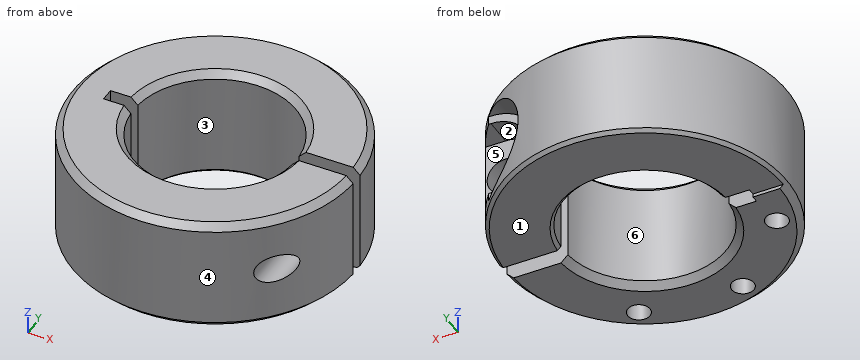
```python
from build123d import *

# Parameters (mm, degrees)
SKETCH2_R             = 21
SKETCH2_R_2           = 12
BOSS_EXTRUDE2_DEPTH   = 17
CHAMFER1_SIZE         = 1
SKETCH3_W             = 46.185652856
SKETCH3_H             = 2
CUT_EXTRUDE1_DEPTH    = 35.219877265
SKETCH5_R             = 2.75
CUT_EXTRUDE3_DEPTH    = 30
CUT_EXTRUDE4_START    = -8
CUT_EXTRUDE4_DEPTH    = 30
M5_TAPPED_HOLE1_D     = 4.2
SKETCH9_W             = 59.171214414
SKETCH9_H             = 29.501144874
CUT_EXTRUDE5_DEPTH    = 0.5
M4_TAPPED_HOLE1_D     = 3.3
M4_TAPPED_HOLE1_DEPTH = 10.1
M4_TAPPED_HOLE1_TIP   = 0.991420021
SKETCH13_R            = 7
CUT_EXTRUDE7_DEPTH    = 17


with BuildPart() as part:
    # Sketch2 → Boss-Extrude2 (new body)
    with BuildSketch(Plane.XY):
        Circle(SKETCH2_R)
        Circle(SKETCH2_R_2, mode=Mode.SUBTRACT)
    extrude(amount=BOSS_EXTRUDE2_DEPTH)

    # Chamfer1
    chamfer1_edges = [part.edges().sort_by_distance(p)[0] for p in [
        (-21, 0, 0),
        (-21, 0, 17),
        (-12, 0, 0),
        (-12, 0, 17),
    ]]
    chamfer(chamfer1_edges, length=CHAMFER1_SIZE)

    # Sketch3 → Cut-Extrude1 (cut, through all)
    with BuildSketch(Plane.XY.offset(17)):
        with Locations((7.092826428, 0)):
            Rectangle(SKETCH3_W, SKETCH3_H)
    extrude(amount=-CUT_EXTRUDE1_DEPTH, mode=Mode.SUBTRACT)

    # Sketch5 → Cut-Extrude3 (cut)
    with BuildSketch(Plane.XZ.offset(-1)):
        with Locations(Location((15.988088482, 8.75, 0), (0, 0, 270))):
            Circle(SKETCH5_R)
    extrude(amount=-CUT_EXTRUDE3_DEPTH, mode=Mode.SUBTRACT)

    # Sketch6 → Cut-Extrude4 (cut)
    with BuildSketch(Plane.XZ.offset(-1).offset(CUT_EXTRUDE4_START)):
        with BuildLine():
            Line((15.988088482, 14.5), (20.976176963, 14.5))
            Line((20.976176963, 14.5), (20.976176963, 3))
            Line((20.976176963, 3), (15.988088482, 3))
            ThreePointArc((15.988088482, 3), (10.238088482, 8.75), (15.988088482, 14.5))
        make_face()
    extrude(amount=-CUT_EXTRUDE4_DEPTH, mode=Mode.SUBTRACT)

    # M5 Tapped Hole1 (through all)
    with Locations(Plane(origin=(0, -1, 0), x_dir=(1, 0, 0), z_dir=(0, 1, 0))):
        with Locations((15.988088482, -8.75)):
            Hole(M5_TAPPED_HOLE1_D / 2)

    # Sketch9 → Cut-Extrude5 (cut)
    with BuildSketch(Plane(origin=(0, 0, 0), x_dir=(-1, 0, 0), z_dir=(0, 0, -1))):
        with Locations((-1.080150951, 14.750572437)):
            Rectangle(SKETCH9_W, SKETCH9_H)
    extrude(amount=-CUT_EXTRUDE5_DEPTH, mode=Mode.SUBTRACT)

    # M4 Tapped Hole1
    with Locations(Plane(origin=(0, 0, 0), x_dir=(-1, 0, 0), z_dir=(0, 0, -1))):
        with Locations((16.444620864, -5.985352508), (-8.75, -15.155444566), (5.985352508, -16.444620864)):
            Hole(M4_TAPPED_HOLE1_D / 2, depth=M4_TAPPED_HOLE1_DEPTH)
            with Locations((0, 0, -(M4_TAPPED_HOLE1_DEPTH + M4_TAPPED_HOLE1_TIP / 2))):  # 118° drill point
                Cone(0, M4_TAPPED_HOLE1_D / 2, M4_TAPPED_HOLE1_TIP, mode=Mode.SUBTRACT)

    # Sketch13 → Cut-Extrude7 (cut)
    with BuildSketch(Plane(origin=(0, 13.2, 0), x_dir=(1, 0, 0), z_dir=(0, 1, 0))):
        with Locations((15.988088482, -8.75)):
            Circle(SKETCH13_R)
    extrude(amount=CUT_EXTRUDE7_DEPTH, mode=Mode.SUBTRACT)


solid = part.part
```
Can you work these out from the model? Positions are in its coordinate system, mm. Face numbers are marked on the shaded views. A direction names the side the tool comes from. Round coordinates to 2 decimals unless told otherwise and drop trailing zeros. Loops run counter-clockwise (first coordinate to the right, second up) from the corner with the lowest first, then second, coordinate; pieces in that order, holes last. Notation, with made-up numbers: (-13.5, 40) -> (43.5, 40) arc R24 ccw to (43.5, 77) -> close; hole circle Ø1 at (11.25, 68). An arc over 180 degrees is marked (long way). Answer in a Markdown table with one row per item.
Item 1: Suppose I cut it at B-B, the plane z = 8.75. List the corners of the cut face in (x, y) for me, plus the area to 3 significant figures.
Answer block:
| item | result |
|---|---|
| outline | (-16, -1) -> (-16, 1) -> (-11.96, 1) arc R12 cw to (11.96, 1) -> (13.24, 1) -> (13.24, 9) -> (10.24, 9) -> (10.24, 13.2) -> (8.99, 13.2) -> (8.99, 18.98) arc R21 ccw (long way) to (13.89, -15.75) -> (13.89, -1) -> (11.96, -1) arc R12 cw to (-11.96, -1) -> close; (18.09, -10.67) arc R21 ccw to (20.98, -1) -> (18.09, -1) -> close; (18.74, 1) -> (20.98, 1) arc R21 ccw to (18.97, 9) -> (18.74, 9) -> close; hole circle Ø3.3 at (-16.44, -5.99); hole circle Ø3.3 at (-5.99, -16.44); hole circle Ø3.3 at (8.75, -15.16) |
| area | 729 mm² |
Item 2: We'd pull the mould along X, two halves only. Please class the marked faces 4, 5 and 6: released by +X, released by -X, zero draft, split by the parting line, or undercut.
Answer block:
| item | result |
|---|---|
| face 4 | split by the parting line |
| face 5 | zero draft |
| face 6 | undercut |
Item 3: If I drill on probe 1 along Y at (x, z) = (-5.5, 4.5); probe 2 along Y at (x, z) = (-15.5, 8.5); probe 3 along X at (y, z) = (3.5, 10.75), over which ranges is the centre line in solid material (lowest first)?
Answer block:
| item | result |
|---|---|
| probe 1 | -20.27 to -18.02, -14.87 to -10.67, 10.67 to 20.27 |
| probe 2 | -14.17 to -7.34, -4.63 to -1, 1 to 14.17 |
| probe 3 | -20.71 to -11.48, 11.48 to 14.1, 17.88 to 20.71 |
Item 4: Suppose I cut it at A-A, the plane x = 0. List the corners of the cut face in (y, z) for me.
Answer block:
| item | result |
|---|---|
| outline | (-21, 1) -> (-20, 0) -> (-13, 0) -> (-12, 1) -> (-12, 16) -> (-13, 17) -> (-20, 17) -> (-21, 16) -> close; (12, 1) -> (12.5, 0.5) -> (20.5, 0.5) -> (21, 1) -> (21, 16) -> (20, 17) -> (13, 17) -> (12, 16) -> close |
Item 5: Suppose I cut it at C-C, the plane z = 12.25. List the corners of the cut face in (x, y) for me, plus the area to 3 significant figures.
Answer block:
| item | result |
|---|---|
| outline | (-16, -1) -> (-16, 1) -> (-11.96, 1) arc R12 cw to (11.96, 1) -> (20.98, 1) arc R21 ccw to (18.97, 9) -> (11.43, 9) -> (11.43, 13.2) -> (9.93, 13.2) -> (9.93, 18.51) arc R21 ccw (long way) to (20.98, -1) -> (11.96, -1) arc R12 cw to (-11.96, -1) -> close |
| area | 861 mm² |
Item 6: On a 3-axis mill with a long thin cutter (end or side, diameter ignored), from which of +Z, -Z, +X, -X, +Y, -Y can I reach the whole of each face in a straight line? I mean the marked faces 1, 2 and 3. Say none if no direction works.
Answer block:
| item | result |
|---|---|
| face 1 | -Z, +X, -X, +Y |
| face 2 | +X, +Y |
| face 3 | +Z, -Z |
Item 7: Will these pins go through, and if not, where does the flat tip stop? P1, Ø3, axis at y = -5, z = 13, coming from the -X side; P2, Ø9.5, axis at x = 16, z = 7.5, coming from the +Y side; P3, Ø6, axis at x = 4, z = 9.5, coming from the -Y side; P4, Ø3.5, axis at x = 15.99, z = 8.75, coming from the +Y side.
Answer block:
| item | result |
|---|---|
| P1 | x = -20.71 |
| P2 | y = 13.2 |
| P3 | y = -20.98 |
| P4 | through |
